from build123d import *

# Parameters (mm, degrees)
FILLET1_R          = 0.4
FILLET2_R          = 0.4
SKETCH3_W          = 0.8
SKETCH3_H          = 1.8
CUT_EXTRUDE1_DEPTH = 5


with BuildPart() as part:
    # Sketch1 → Revolve1 (revolve)
    with BuildSketch(Plane.XY, mode=Mode.PRIVATE) as revolve1_sk:
        with BuildLine():
            Line((0, 0), (-1.5, 0))
            Line((-1.5, 0), (-1.5, 3))
            Line((-1.5, 3), (-2.5, 3))
            Line((-2.5, 3), (-2.5, 6.856465997))
            ThreePointArc((-2.5, 6.856465997), (-1.595582496, 7.695582496), (-0.4, 8))
            Line((-0.4, 8), (0, 8))
            Line((0, 8), (0, 5.056465997))
            Line((0, 5.056465997), (0, 0))
        make_face()
    revolve(revolve1_sk.sketch.rotate(Axis((0, 5.056465997, 0), (0, -1, 0)), 270), axis=Axis((0, 5.056465997, 0), (0, -1, 0)))

    # Fillet1
    fillet1_edges = [part.edges().sort_by_distance(p)[0] for p in [
        (0, 3, -1.5),
    ]]
    fillet(fillet1_edges, radius=FILLET1_R)

    # Fillet2
    fillet2_edges = [part.edges().sort_by_distance(p)[0] for p in [
        (0, 0, -1.5),
    ]]
    fillet(fillet2_edges, radius=FILLET2_R)

    # Sketch3 → Cut-Extrude1 (cut, symmetric)
    with BuildSketch(Plane.XY):
        with Locations((0, 7.1)):
            Rectangle(SKETCH3_W, SKETCH3_H)
    extrude(amount=CUT_EXTRUDE1_DEPTH, both=True, mode=Mode.SUBTRACT)


solid = part.part
Here's how the part is built. I have some questions about the finished solid (model axes, mm). A direction names the side the tool comes from. Coordinates: 2 decimals unless noted, no trailing zeros. Order: outer loops, then holes, each group sorted by start corner. A loop starts at its lowest first (then second) coordinate and runs counter-clockwise, first axis right, second up. Notation, with made-up numbers: (11.25, 54.5) - (26.25, 54.5) arc R22 cw to (26.25, 75.5) - close; hole circle Ø10 at (30.5, -32). An arc over 180 degrees is marked (long way). Use CSV: the item, a comma, the result in double quotes. Start each with the question number.
1. For faces 4 (the face through (-1, 3, -2)), 5 (the face through (0.4, 7, 0)), 6 (the face through (-0.751, 4.955, 2.385)), which set-ups out of +Z, -Z, +X, -X, +Y, -Y let a thin tool reach every point of the face, with its end or its side?
2. Suppose I cut it at A-A on x = 0. List the corners of the cut face in (y, z) for me, then the cut area to 3 significant figures.
3. Suppose I cut it at B-B on y = 5.25. List the corners of the cut face in (x, z) for me.
4. If we mould it in two halves opening along X, with no side actions, what happens to faces 1 (the face through (0, 0, 0)), 2 (the face through (0, 6.2, 0)), 3 (the face through (-0.45, 1.52, 1.43))? For each: +X half, -X half, draft (parallel to the pull), parting line (faces both ways), or undercut.
5. I'm going to push flat-ended pins straight in: pin 1 (2 mm diameter, centred on x = -1.5, y = 4.5, fed in from -Z); pin 2 (1.5 mm diameter, centred on x = 0.5, z = -0.5, fed in from -Y); pin 3 (0.9 mm diameter, centred on x = 0, z = 1, fed in from +Y); pin 4 (2 mm diameter, centred on y = 7.5, z = -1, fed in from +X). Where does each tip first touch, or does it pass through?
6. Suppose I cut it at C-C on y = 0.75. List the corners of the cut face in (x, z) for me, then the cut area to 3 significant figures.
7. Please list where these lines run through material, in increasing order: line 1 (X direction, y = 6.25, z = 0.55); line 2 (Y direction, x = 0.2, z = -0.1); line 3 (X direction, y = 7, z = -1.35). Write a range as from..to.
Output:
1,face 4,"-Y"
1,face 5,"+Z, -Z, +Y"
1,face 6,"+Y, -Y"
2,outline,"(0, -1.1) arc R0.4 ccw to (0.4, -1.5) - (2.6, -1.5) arc R0.4 cw to (3, -1.9) - (3, -2.5) - (6.2, -2.5) - (6.2, 2.5) - (3, 2.5) - (3, 1.9) arc R0.4 cw to (2.6, 1.5) - (0.4, 1.5) arc R0.4 ccw to (0, 1.1) - close"
2,area,"25.0 mm2"
3,outline,"circle Ø5 at (0, 0)"
4,face 1,"draft"
4,face 2,"undercut"
4,face 3,"parting line"
5,pin 1,"stops at z = -2.45"
5,pin 2,"stops at y = 0"
5,pin 3,"stops at y = 7.95"
5,pin 4,"stops at x = 2.49"
6,outline,"circle Ø3 at (0, 0)"
6,area,"7.07 mm2"
7,line 1,"x = -2.44..-0.4, 0.4..2.44"
7,line 2,"y = 0..6.2"
7,line 3,"x = -1.98..-0.4, 0.4..1.98"
